Geometry check sheet. Reference: drawing and pictorial views, mm from the part's lowest x, y, z. Coordinates: 2 decimals unless noted, no trailing zeros. Write each loop counter-clockwise with the first axis right and the second up, starting at its lowest first coordinate (ties: lowest second). Pieces come first, ordered by that corner, then holes. Notation, with made-up numbers: (53, 19) -> (93, 19) arc R17 ccw to (93, 42) -> close; hole circle Ø10 at (-38.5, -6.5). An arc over 180 degrees is marked (long way). Answer in a Markdown table with one row per item.
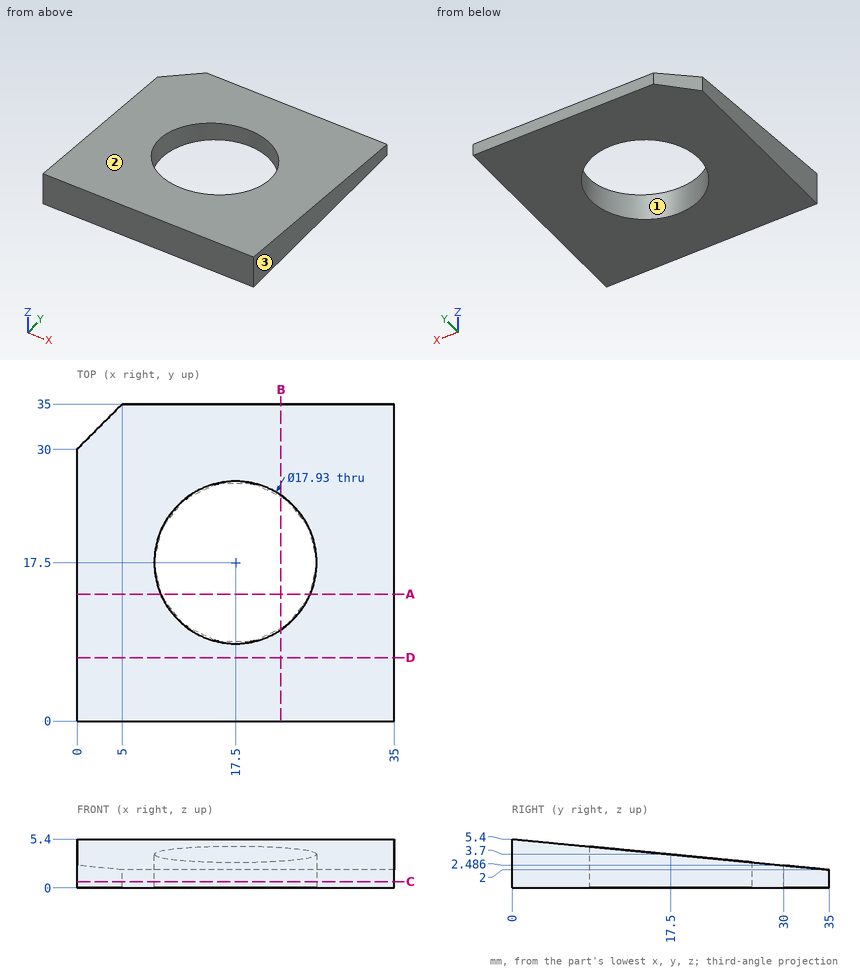
1. Depth check by flat-ended pin: P1, Ø5, axis at x = 5, y = 16.5, coming from the -Z side. Enter the tip coordinate at first touch or a pass-through.
Geometry says:
| item | result |
|---|---|
| P1 | z = 0 |
2. Section check A-A, the plane y = 14. Record the boundary of the cut face in (x, z).
Geometry says:
| item | result |
|---|---|
| outline | (0, 0) -> (9.25, 0) -> (9.25, 4.04) -> (0, 4.04) -> close; (25.75, 0) -> (35, 0) -> (35, 4.04) -> (25.75, 4.04) -> close |
3. Section check B-B, the plane x = 22.5. Record the boundary of the cut face in (y, z).
Geometry says:
| item | result |
|---|---|
| outline | (0, 0) -> (10.06, 0) -> (10.06, 4.42) -> (0, 5.4) -> close; (24.94, 0) -> (35, 0) -> (35, 2) -> (24.94, 2.98) -> close |
4. Section check D-D, the plane y = 7. Record the boundary of the cut face in (x, z), plus the area to 3 significant figures.
Geometry says:
| item | result |
|---|---|
| outline | (0, 0) -> (35, 0) -> (35, 4.72) -> (0, 4.72) -> close |
| area | 165 mm^2 |
5. Mould release check, pull along Y, two halves, no side actions. Record for the marked faces 1, 2 and 3: released by +Y, released by -Y, zero draft, split by the parting line, or undercut.
Geometry says:
| item | result |
|---|---|
| face 1 | undercut |
| face 2 | released by +Y |
| face 3 | zero draft |
6. Thickness scan on line 1 (X direction, y = 17.5, z = 3.1) (1 decimal); line 2 (X direction, y = 23, z = 2.55). Record the ranges inside material, lowest first. Write a range as from..to.
Geometry says:
| item | result |
|---|---|
| line 1 | 0..8.5, 26.5..35 |
| line 2 | 0..10.42, 24.58..35 |
7. Section check C-C, the plane z = 0.7. Record the boundary of the cut face in (x, y) (1 decimal).
Geometry says:
| item | result |
|---|---|
| outline | (0, 0) -> (35, 0) -> (35, 35) -> (5, 35) -> (0, 30) -> close; hole circle Ø17.9 at (17.5, 17.5) |
